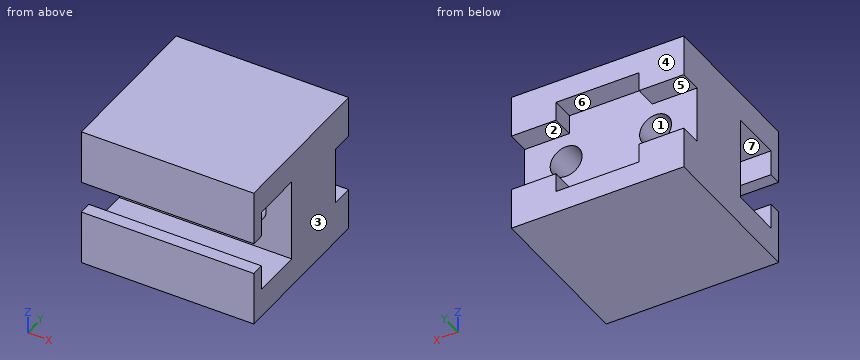
```python
from build123d import *

# Parameters (mm, degrees)
BASE_BLOCK_SKETCH_W       = 54
BASE_BLOCK_SKETCH_H       = 50
BASE_BLOCK_54X50X44_DEPTH = 44
TOP_POCKET_7_DEEP_DEPTH   = 7
T_SLOT_CUT_DEPTH          = 75.006756448
POCKET_HOLES_SKETCH_R     = 5
POCKET_HOLES_2X_10_DEPTH  = 68.186308129


with BuildPart() as part:
    # Base Block Sketch → Base Block 54x50x44 (new body)
    with BuildSketch(Plane.XY):
        Rectangle(BASE_BLOCK_SKETCH_W, BASE_BLOCK_SKETCH_H)
    extrude(amount=-BASE_BLOCK_54X50X44_DEPTH)

    # Top Pocket Sketch → Top Pocket 7 Deep (cut)
    with BuildSketch(Plane(origin=(0, 25, 0), x_dir=(1, 0, 0), z_dir=(0, 1, 0))):
        Polygon((-13, 37), (13, 37), (13, 31), (27, 31), (27, 13), (13, 13), (13, 7), (-13, 7), (-13, 13), (-27, 13), (-27, 31), (-13, 31), align=None)
    extrude(amount=-TOP_POCKET_7_DEEP_DEPTH, mode=Mode.SUBTRACT)

    # T-Slot Sketch → T-Slot Cut (cut, through all)
    with BuildSketch(Plane.ZY.offset(27)):
        Polygon((-27, -25), (-27, -21), (-35, -21), (-35, -5), (-9, -5), (-9, -21), (-17, -21), (-17, -25), align=None)
    extrude(amount=-T_SLOT_CUT_DEPTH, mode=Mode.SUBTRACT)

    # Pocket Holes Sketch → Pocket Holes 2xØ10 (cut, through all)
    with BuildSketch(Plane(origin=(0, 18, 0), x_dir=(1, 0, 0), z_dir=(0, 1, 0))):
        with Locations(Location((-14, 22, 0), (0, 0, 270))):
            Circle(POCKET_HOLES_SKETCH_R)
        with Locations(Location((14, 22, 0), (0, 0, 270))):
            Circle(POCKET_HOLES_SKETCH_R)
    extrude(amount=-POCKET_HOLES_2X_10_DEPTH, mode=Mode.SUBTRACT)


solid = part.part
```
Work out the finished part from the listing and answer in its coordinate system (mm). Face numbers are marked on the shaded views. A direction names the side the tool comes from. Give positions to 0.01 mm unless a question says otherwise; leave off trailing zeros. Loops run counter-clockwise (first coordinate to the right, second up) from the corner with the lowest first, then second, coordinate; pieces in that order, holes last. Notation, with made-up numbers: (31, 33) -> (58, 33) arc R14 cw to (58, 46) -> close; hole circle Ø1 at (41, -23). An arc over 180 degrees is marked (long way). Write item = value, one per line. Start each with the question number.
(1) Find section D-D on y = 14.5. Give the vertices of the cut face in (x, z), and give its area (3 significant figures).
(2) Find the intervals of material crossed by probe 1 along X at (y, z) = (3.75, -22); probe 2 along Z at (x, y) = (22, -8); probe 3 along Z at (x, y) = (-2.5, -22), in increasing order. Write a range as from..to.
(3) Find section B-B on z = -19. Give the vertices of the cut face in (x, y).
(4) Find section C-C on x = -14. Give the vertices of the cut face in (y, z).
(5) Which of the six approach directions +Z, -Z, +X, -X, +Y, -Y give full straight-line access (tool end or side, diameter ignored) to the marked faces 4, 5, 6 and 7?
(6) Given pin 1 Ø1 at (x, y) = (4, -9) entering from +Z; pin 2 Ø12 at (x, z) = (-10.5, -21.5) entering from +Y, each flat-ended and moving along its own axis, determine where each tip first touches the part or whether it passes through.
(7) The mould has two halves that part along X. Classify the marked faces 1, 2 and 3: +X half, -X half, draft (parallel to the pull), parting line (faces both ways), or undercut.
(8) Find section A-A on z = -10. Give the vertices of the cut face in (x, y).
From the geometry:
q1.outline = (-27, -44) -> (27, -44) -> (27, 0) -> (-27, 0) -> close; hole circle Ø10 at (-14, -22); hole circle Ø10 at (14, -22)
q1.area = 2,220 mm^2
q2.probe_1 = -27..-19, -9..9, 19..27
q2.probe_2 = -44..-35, -9..0
q2.probe_3 = -44..-27, -17..0
q3.outline = (-27, -5) -> (-18, -5) -> (-18, 18) -> (-27, 18) -> close; (-10, -5) -> (10, -5) -> (10, 18) -> (-10, 18) -> close; (18, -5) -> (27, -5) -> (27, 18) -> (18, 18) -> close
q4.outline = (-25, -44) -> (25, -44) -> (25, -31) -> (18, -31) -> (18, -27) -> (-5, -27) -> (-5, -35) -> (-21, -35) -> (-21, -27) -> (-25, -27) -> close; (-25, -17) -> (-21, -17) -> (-21, -9) -> (-5, -9) -> (-5, -17) -> (18, -17) -> (18, -13) -> (25, -13) -> (25, 0) -> (-25, 0) -> close
q5.face_4 = +Z, -Z, +X, -X, +Y
q5.face_5 = +X, -X, +Y
q5.face_6 = +Y
q5.face_7 = +X, -X
q6.pin_1 = 0
q6.pin_2 = 18
q7.face_1 = undercut
q7.face_2 = draft
q7.face_3 = +X half
q8.outline = (-27, -25) -> (27, -25) -> (27, -21) -> (-27, -21) -> close; (-27, -5) -> (27, -5) -> (27, 25) -> (13, 25) -> (13, 18) -> (-13, 18) -> (-13, 25) -> (-27, 25) -> close
